Geometry check sheet. Reference: the model listing, model coordinates, mm. Face numbers are marked on the shaded views. A direction names the side the tool comes from. Round coordinates to 2 decimals unless told otherwise and drop trailing zeros. Write each loop counter-clockwise with the first axis right and the second up, starting at its lowest first coordinate (ties: lowest second). Pieces come first, ordered by that corner, then holes.
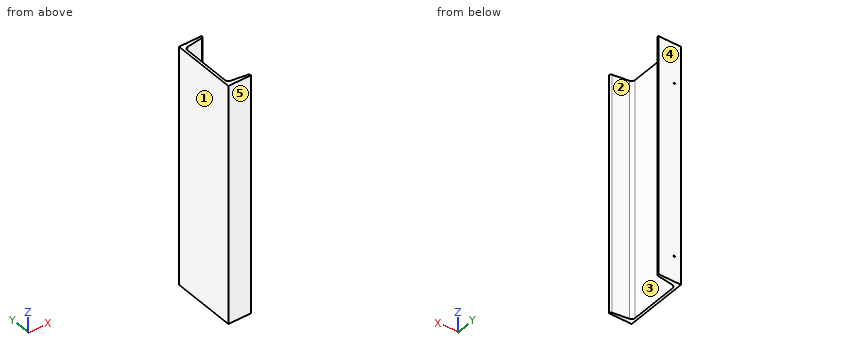
from build123d import *

# Parameters (mm, degrees)
EXTRUDE_1_DEPTH        = 895
HOLE_WIZARD_M6_1_D     = 5
HOLE_WIZARD_M6_1_DEPTH = 15
HOLE_WIZARD_M6_1_TIP   = 1.502151548


with BuildPart() as part:
    # 草图1 → 凸台-拉伸1 (new body)
    with BuildSketch(Plane.XY):
        with BuildLine():
            Line((0, 0), (-85, 0))
            Line((-85, 0), (-85, -240))
            Line((-85, -240), (0, -240))
            Line((0, -240), (0, -238.623349271))
            ThreePointArc((0, -238.623349271), (-1.594387729, -234.358965582), (-5.595374844, -232.186606824))
            Line((-5.595374844, -232.186606824), (-64.309250312, -223.934909757))
            ThreePointArc((-64.309250312, -223.934909757), (-72.311224543, -219.59019224), (-75.5, -211.061424863))
            Line((-75.5, -211.061424863), (-75.5, -28.938575137))
            ThreePointArc((-75.5, -28.938575137), (-72.311224543, -20.40980776), (-64.309250312, -16.065090243))
            Line((-64.309250312, -16.065090243), (-5.595374844, -7.813393176))
            ThreePointArc((-5.595374844, -7.813393176), (-1.594387729, -5.641034418), (0, -1.376650729))
            Line((0, -1.376650729), (0, 0))
        make_face()
    extrude(amount=EXTRUDE_1_DEPTH)

    # M6 螺纹孔1
    with Locations(Plane(origin=(0, 0, 0), x_dir=(1, 0, 0), z_dir=(0, 1, 0))):
        with Locations((-60, -745), (-60, -95)):
            Hole(HOLE_WIZARD_M6_1_D / 2, depth=HOLE_WIZARD_M6_1_DEPTH)
            with Locations((0, 0, -(HOLE_WIZARD_M6_1_DEPTH + HOLE_WIZARD_M6_1_TIP / 2))):  # 118° drill point
                Cone(0, HOLE_WIZARD_M6_1_D / 2, HOLE_WIZARD_M6_1_TIP, mode=Mode.SUBTRACT)


solid = part.part
1. Scan lines: line 1 along Z through (x, y) = (-60, -4); line 2 along Y through (x, z) = (-16.5, 68); line 3 along Y through (x, z) = (-27, 86). Record each from-to range of solid material in increasing order.
2. Release check for a two-part mould opening along Y. For the marked faces 3, 4 and 5 record: +Y half, -Y half, draft (parallel to the pull), parting line (faces both ways), or undercut.
3. Section check C-C (y = -76.5). Record the cut outline in (x, z).
4. Access from +Z, -Z, +X, -X, +Y, -Y to the whole of each face (thin tool, end or side, straight path). Record for the marked faces 1 and 2.
5. Section check A-A (x = -25). Record the cut outline in (y, z), plus the area to 3 significant figures.
6. Section check B-B (z = 425). Record the cut outline in (x, y).
7. Depth check by flat-ended pin: pin 1 Ø2 at (y, z) = (-157, 477) entering from +X; pin 2 Ø12 at (y, z) = (-208.5, 666.5) entering from +X. Enter the tip coordinate at first touch or a pass-through.
Results below:
1. line 1: z = 0 to 92.5, 97.5 to 742.5, 747.5 to 895
1. line 2: y = -240 to -230.65, -9.35 to 0
1. line 3: y = -240 to -229.18, -10.82 to 0
2. face 3: undercut
2. face 4: +Y half
2. face 5: -Y half
3. outline: (-85, 0) - (-75.5, 0) - (-75.5, 895) - (-85, 895) - close
4. face 1: +Z, -Z, -X, +Y, -Y
4. face 2: +Z, -Z, +X
5. outline: (-240, 0) - (-229.46, 0) - (-229.46, 895) - (-240, 895) - close; (-10.54, 0) - (0, 0) - (0, 895) - (-10.54, 895) - close
5. area: 18,900 mm2
6. outline: (-85, -240) - (0, -240) - (0, -238.62) arc R6.5 ccw to (-5.6, -232.19) - (-64.31, -223.93) arc R13 cw to (-75.5, -211.06) - (-75.5, -28.94) arc R13 cw to (-64.31, -16.07) - (-5.6, -7.81) arc R6.5 ccw to (0, -1.38) - (0, 0) - (-85, 0) - close
7. pin 1: stops at x = -75.5
7. pin 2: stops at x = -75.04
